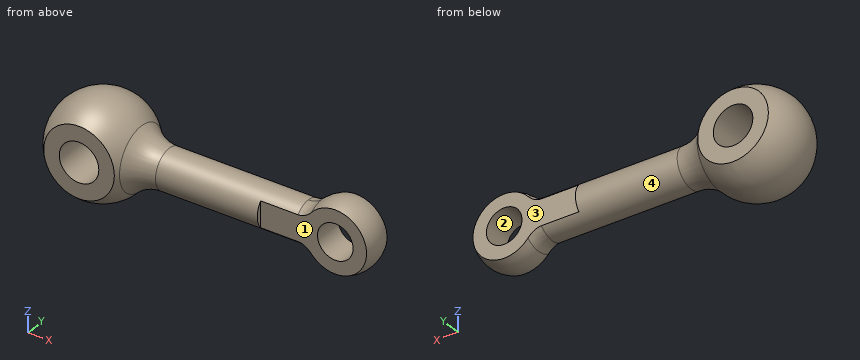
```python
from build123d import *

# Parameters (mm, degrees)
END_BLEND_FILLET_R10_A_R = 10
END_BLEND_FILLET_R10_B_R = 10
SHAFT_FLAT_CUT_REACH     = 101.084
SHAFT_START              = 7.5
SHAFT_FLAT_SKETCH_W      = 28.74
SHAFT_FLAT_SKETCH_H      = 13.228756556


with BuildPart() as part:
    # Rod Revolve Profile → Rod Body Revolve (revolve)
    with BuildSketch(Plane.XY, mode=Mode.PRIVATE) as rod_body_revolve_sk:
        with BuildLine():
            ThreePointArc((-43.496428929, 17.5), (-36.54418797, 11.972243623), (-27.883933933, 10))
            Line((-27.883933933, 10), (52.35, 10))
            Line((52.35, 10), (52.35, 0))
            Line((52.35, 0), (-51.35, 0))
            Line((-51.35, 0), (-51.35, 17.5))
            Line((-51.35, 17.5), (-43.496428929, 17.5))
        make_face()
    revolve(rod_body_revolve_sk.sketch.rotate(Axis((-51.35, 0, 0), (1, 0, 0)), 90), axis=Axis((-51.35, 0, 0), (1, 0, 0)))

    # Sketch5_17 → End Boss Revolve A (revolve)
    with BuildSketch(Plane.XY, mode=Mode.PRIVATE) as end_boss_revolve_a_sk:
        with BuildLine():
            Line((-71.35, 17.5), (-79.203571071, 17.5))
            ThreePointArc((-79.203571071, 17.5), (-86.35, 0), (-79.203571071, -17.5))
            Line((-79.203571071, -17.5), (-71.35, -17.5))
            Line((-71.35, -17.5), (-71.35, 17.5))
        make_face()
    revolve(end_boss_revolve_a_sk.sketch.rotate(Axis((-61.35, -17.5, 0), (0, 1, 0)), 270), axis=Axis((-61.35, -17.5, 0), (0, 1, 0)))

    # Sketch5_18 → End Boss Revolve B (revolve)
    with BuildSketch(Plane.XY, mode=Mode.PRIVATE) as end_boss_revolve_b_sk:
        with BuildLine():
            Line((77.161388301, -7.5), (70.35, -7.5))
            Line((70.35, -7.5), (70.35, 7.5))
            Line((70.35, 7.5), (77.161388301, 7.5))
            ThreePointArc((77.161388301, 7.5), (78.85, 0), (77.161388301, -7.5))
        make_face()
    revolve(end_boss_revolve_b_sk.sketch.rotate(Axis((61.35, 7.5, 0), (0, -1, 0)), 180), axis=Axis((61.35, 7.5, 0), (0, -1, 0)))

    # End Blend Fillet R10 A
    end_blend_fillet_r10_a_edges = [part.edges().sort_by_distance(p)[0] for p in [
        (46.988593384, 4.114378278, 9.114378278),
    ]]
    fillet(end_blend_fillet_r10_a_edges, radius=END_BLEND_FILLET_R10_A_R)

    # End Blend Fillet R10 B
    end_blend_fillet_r10_b_edges = [part.edges().sort_by_distance(p)[0] for p in [
        (46.988593384, 0, -10),
    ]]
    fillet(end_blend_fillet_r10_b_edges, radius=END_BLEND_FILLET_R10_B_R)

    # Shaft Flat Sketch → Shaft Flat Cut (cut, up to next)
    with BuildSketch(Plane(origin=(0, 0, 0), x_dir=(1, 0, 0), z_dir=(0, 1, 0)).offset(SHAFT_START), mode=Mode.PRIVATE) as shaft_flat_cut_sk1:
        with Locations((37.98, 0)):
            Rectangle(SHAFT_FLAT_SKETCH_W, SHAFT_FLAT_SKETCH_H)
    shaft_flat_cut_tool1 = extrude(shaft_flat_cut_sk1.sketch, amount=SHAFT_FLAT_CUT_REACH, mode=Mode.PRIVATE) & part.part
    shaft_flat_cut = shaft_flat_cut_tool1.solids().sort_by_distance((37.98, 7.5, 0))[0]
    add(shaft_flat_cut, mode=Mode.SUBTRACT)

    # Shaft Flat Mirror: Shaft Flat Cut across plane
    add(shaft_flat_cut.mirror(Plane.ZX), mode=Mode.SUBTRACT)


solid = part.part
```
Check sheet for the modelled part. Datum: model origin and axes. Units: mm. Face numbers are marked on the shaded views. A direction names the side the tool comes from. Round coordinates to 2 decimals unless told otherwise and drop trailing zeros. Loops run counter-clockwise (first coordinate to the right, second up) from the corner with the lowest first, then second, coordinate; pieces in that order, holes last. Notation, with made-up numbers: M 72,11 L 126,11 A26 cw 126,31 Z; hole C 36.25,56 d1. An arc over 180 degrees is marked long. Answer as a JSON object with one key per item and string values.
1. Section check B-B (x = 61.35). Record the boundary of the cut face in (y, z), plus the area to 3 significant figures.
Reply:
{"outline": "M -7.5,-15.81 A17.5 ccw 7.5,-15.81 L 7.5,-9 L -7.5,-9 Z; M -7.5,9 L 7.5,9 L 7.5,15.81 A17.5 ccw -7.5,15.81 Z", "area": "238 mm²"}
2. Scan lines: line 1 (Z direction, x = 61.35, y = 1); line 2 (Y direction, x = 41.5, z = -3); line 3 (X direction, y = 12, z = 6). Record each from-to range of solid material in increasing order.
Reply:
{"line 1": "z = -17.47 to -9, 9 to 17.47", "line 2": "y = -7.5 to 7.5", "line 3": "x = -82.45 to -69.35, -53.35 to -39.06"}
3. Section check C-C (x = -61.35). Record the boundary of the cut face in (y, z), plus the area to 3 significant figures.
Reply:
{"outline": "M -17.5,-17.85 A25 ccw 17.5,-17.85 L 17.5,-10 L -17.5,-10 Z; M -17.5,10 L 17.5,10 L 17.5,17.85 A25 ccw -17.5,17.85 Z", "area": "894 mm²"}
4. Mould release check, pull along X, two halves, no side actions. Record for the marked faces 3 and 4: pulls with the +X half, pulls with the -X half, needs draft (parallel to the pull), parting line crosses it, or undercut.
Reply:
{"face 3": "needs draft", "face 4": "undercut"}
5. Section check D-D (y = -5). State how many separate pieces and enclosed holes the cut face has, plus the area to 3 significant figures.
Reply:
{"separate pieces": "1", "enclosed holes": "2", "area": "3,670 mm²"}
6. Gauge pin test, flat ends, axial feed: P1, Ø3, axis at x = 4, z = -7.5, coming from the +Y side; P2, Ø0.8, axis at y = 8.5, z = -1.5, coming from the +X side; P3, Ø4, axis at x = -34, z = -4, coming from the +Y side; P4, Ø23, axis at x = -61.35, z = 0, coming from the -Y side. Record the tip position at first contact, or that the pin passes through.
Reply:
{"P1": "stops at y = 8", "P2": "stops at x = 23.61", "P3": "stops at y = 11.21", "P4": "stops at y = -17.5"}
7. Access from +Z, -Z, +X, -X, +Y, -Y to the whole of each face (thin tool, end or side, straight path). Record for the marked faces 1 and 2.
Reply:
{"face 1": "+Z, -Z, +X, -Y", "face 2": "+Y, -Y"}
8. Section check A-A (z = 0). Record the boundary of the cut face in (x, y), plus the area to 3 significant figures.
Reply:
{"outline": "M -79.2,-17.5 L -71.35,-17.5 L -71.35,17.5 L -79.2,17.5 A25 ccw Z; M -51.35,-17.5 L -43.5,-17.5 A25 ccw -42.01,-15.84 A20 cw -27.88,-10 L 23.61,-10 L 23.61,-7.5 L 52.35,-7.5 L 52.35,7.5 L 23.61,7.5 L 23.61,10 L -27.88,10 A20 cw -42.01,15.84 A25 ccw -43.5,17.5 L -51.35,17.5 Z; M 70.35,-7.5 L 77.16,-7.5 A17.5 ccw 77.16,7.5 L 70.35,7.5 Z", "area": "2,690 mm²"}
